from build123d import *

# Parameters (mm, degrees)
SKETCH_1_W             = 60
SKETCH_1_H             = 73
SKETCH_1_R             = 20
EXTRUDE_1_DEPTH        = 7
EXTRUDE_START          = -2
SKETCH_2_R             = 20
SKETCH_2_R_2           = 18.5
EXTRUDE_2_DEPTH        = 2
CHAMFER_1_SIZE         = 10
HOLE_WIZARD_M6_1_D     = 5
HOLE_WIZARD_M6_1_DEPTH = 14
HOLE_WIZARD_M6_1_TIP   = 1.502151548


with BuildPart() as part:
    # 草图1 → 凸台-拉伸1 (new, symmetric)
    with BuildSketch(Plane.XY):
        Rectangle(SKETCH_1_W, SKETCH_1_H)
        with Locations((0, 6.5)):
            Circle(SKETCH_1_R, mode=Mode.SUBTRACT)
    extrude(amount=EXTRUDE_1_DEPTH, both=True)

    # 草图2 → 凸台-拉伸2 (add)
    with BuildSketch(Plane.XY.offset(7).offset(EXTRUDE_START)):
        with Locations((0, 6.5)):
            Circle(SKETCH_2_R)
        with Locations((0, 6.5)):
            Circle(SKETCH_2_R_2, mode=Mode.SUBTRACT)
    extrude(amount=EXTRUDE_2_DEPTH)

    # 倒角1
    chamfer_1_edges = [part.edges().sort_by_distance(p)[0] for p in [
        (-30, 36.5, 0),
        (30, 36.5, 0),
    ]]
    chamfer(chamfer_1_edges, length=CHAMFER_1_SIZE)

    # M6 螺纹孔1
    with Locations(Plane(origin=(-24, -36.5, 0), x_dir=(0, 0, -1), z_dir=(0, -1, 0))):
        with Locations((0, 0), (0, 48)):
            Hole(HOLE_WIZARD_M6_1_D / 2, depth=HOLE_WIZARD_M6_1_DEPTH)
            with Locations((0, 0, -(HOLE_WIZARD_M6_1_DEPTH + HOLE_WIZARD_M6_1_TIP / 2))):  # 118° drill point
                Cone(0, HOLE_WIZARD_M6_1_D / 2, HOLE_WIZARD_M6_1_TIP, mode=Mode.SUBTRACT)


solid = part.part
The listing builds one solid part. Answer for the finished solid, in the listing's coordinates (mm). A direction names the side the tool comes from. Coordinates: 2 decimals unless noted, no trailing zeros. Order: outer loops, then holes, each group sorted by start corner. A loop starts at its lowest first (then second) coordinate and runs counter-clockwise, first axis right, second up.
Q1. For a pull along Z with two mould halves and no side action, classify faces 4 (the face through (-21.52, -29.4, -0.33)), 5 (the face through (-30, -5, 0)), 6 (the face through (0, -16, -7)) as pulls with the +Z half, pulls with the -Z half, needs draft (parallel to the pull), parting line crosses it, or undercut.
Q2. A cutting plane is placed at A-A, the plane y = 6.5. Write down the section's boundary in (x, z), and give its area (3 significant figures).
Q3. Consider line 1 (X direction, y = -28.25, z = 0); line 2 (Y direction, x = 0, z = 1); line 3 (Z direction, x = 24, y = -27). Determine where each line is inside the solid, lowest interval first.
Q4. Which of the six approach directions +Z, -Z, +X, -X, +Y, -Y give full straight-line access (tool end or side, diameter ignored) to faces 1 (the face through (26.48, -29.4, -0.33)), 2 (the face through (0, -36.5, 0)), 3 (the face through (18, 1, 5))?
Q5. A cutting plane is placed at B-B, the plane x = 0. Write down the section's boundary in (y, z).
Q6. A cutting plane is placed at C-C, the plane z = -3.5. Write down the section's boundary in (x, y), and give its area (3 significant figures).
Q7. Given P1, Ø1, axis at x = 3.5, y = 23.5, coming from the -Z side, flat-ended and moving along its own axis, determine where the tip first touches the part or whether it passes through.
Q8. A cutting plane is placed at D-D, the plane y = -23.5. Write down the section's boundary in (x, z), and give its area (3 significant figures).
Answers follow:
1. face 4: undercut
1. face 5: needs draft
1. face 6: pulls with the -Z half
2. outline: (-30, -7) - (-20, -7) - (-20, 5) - (-18.5, 5) - (-18.5, 7) - (-30, 7) - close; (18.5, 5) - (20, 5) - (20, -7) - (30, -7) - (30, 7) - (18.5, 7) - close
2. area: 286 mm2
3. line 1: x = -30 to -26.5, -21.5 to 21.5, 26.5 to 30
3. line 2: y = -36.5 to -13.5, 26.5 to 36.5
3. line 3: z = -7 to -2.5, 2.5 to 7
4. face 1: -Y
4. face 2: +Z, -Z, +X, -X, -Y
4. face 3: -Z
5. outline: (-36.5, -7) - (-13.5, -7) - (-13.5, 5) - (-12, 5) - (-12, 7) - (-36.5, 7) - close; (25, 5) - (26.5, 5) - (26.5, -7) - (36.5, -7) - (36.5, 7) - (25, 7) - close
6. outline: (-30, -36.5) - (30, -36.5) - (30, 26.5) - (20, 36.5) - (-20, 36.5) - (-30, 26.5) - close; hole circle Ø40 at (0, 6.5)
6. area: 3,020 mm2
7. P1: passes through
8. outline: (-30, -7) - (30, -7) - (30, 7) - (-30, 7) - close; hole circle Ø5 at (-24, 0); hole circle Ø5 at (24, 0)
8. area: 801 mm2
